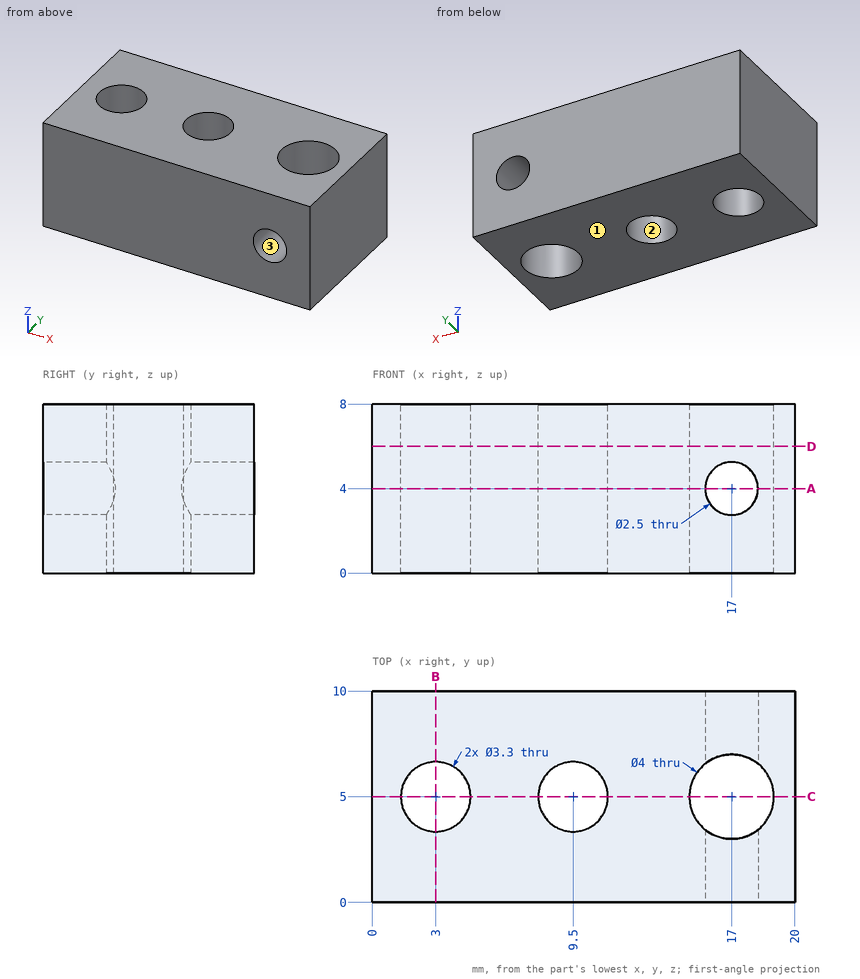
Job drawing, mm, ordinate dimensions from the low corner. One solid piece. Give positions to 0.01 mm unless a question says otherwise; leave off trailing zeros. Write each loop counter-clockwise with the first axis right and the second up, starting at its lowest first coordinate (ties: lowest second). Pieces come first, ordered by that corner, then holes. Notation, with made-up numbers: M -0.75,48.5 L 9.25,48.5 A22 ccw 9.25,80.5 Z; hole C 38,46 d8. An arc over 180 degrees is marked long. One line per item, written item: value. Start each with the question number.
Q1. Saw through at A-A, the plane z = 4. Write the cut outline in (x, y).
Q2. Saw through at B-B, the plane x = 3. Write the cut outline in (y, z).
Q3. Saw through at C-C, the plane y = 5. Write the cut outline in (x, z), plus the area to 3 significant figures.
Q4. Two-plate mould, pull along Z, no slides. Class the marked faces 1, 2 and 3: +Z half, -Z half, draft (parallel to the pull), parting line (faces both ways), or undercut.
Q5. Probe probe 1 along Y at (x, z) = (9.5, 4.75); probe 2 along Z at (x, y) = (17, 1.65); probe 3 along Y at (x, z) = (17, 2.5). List the from-to ranges inside material, lowest first. Write a range as [from, to].
Q6. Saw through at D-D, the plane z = 6. Write the cut outline in (x, y), plus the area to 3 significant figures.
Q7. Drop a flat-ended pin along its axis: pin 1 Ø3.5 at (x, y) = (17, 5) entering from -Z. Give the stop position or say it passes through.
Output values:
1. outline: M 0,0 L 15.75,0 L 15.75,3.44 A2 cw 15.75,6.56 L 15.75,10 L 0,10 Z; M 18.25,0 L 20,0 L 20,10 L 18.25,10 L 18.25,6.56 A2 cw 18.25,3.44 Z; hole C 3,5 d3.3; hole C 9.5,5 d3.3
2. outline: M 0,0 L 3.35,0 L 3.35,8 L 0,8 Z; M 6.65,0 L 10,0 L 10,8 L 6.65,8 Z
3. outline: M 0,0 L 1.35,0 L 1.35,8 L 0,8 Z; M 4.65,0 L 7.85,0 L 7.85,8 L 4.65,8 Z; M 11.15,0 L 15,0 L 15,8 L 11.15,8 Z; M 19,0 L 20,0 L 20,8 L 19,8 Z
3. area: 75.2 mm²
4. face 1: -Z half
4. face 2: draft
4. face 3: undercut
5. probe 1: y = [0, 3.35], [6.65, 10]
5. probe 2: z = [0, 2.75], [5.25, 8]
5. probe 3: y = [0, 3], [7, 10]
6. outline: M 0,0 L 20,0 L 20,10 L 0,10 Z; hole C 3,5 d3.3; hole C 9.5,5 d3.3; hole C 17,5 d4
6. area: 170 mm²
7. pin 1: passes through
